CAD build for the part. Positions are in the model's coordinates, mm. A direction names the side the tool comes from. Give positions to 0.01 mm unless a question says otherwise; leave off trailing zeros. Order: outer loops, then holes, each group sorted by start corner. A loop starts at its lowest first (then second) coordinate and runs counter-clockwise, first axis right, second up. Notation, with made-up numbers: (71, 4) -> (79, 4) arc R18 cw to (79, 13) -> close; hole circle Ø2 at (43, -7.5). An arc over 180 degrees is marked (long way). Answer as CSV lines item,"result".
```python
from build123d import *

# Parameters (mm, degrees)
SKETCH_1_R          = 15
EXTRUDE_1_DEPTH     = 50
SKETCH_2_R          = 20
EXTRUDE_2_DEPTH     = 15
SKETCH_3_W          = 60.184655206
SKETCH_3_H          = 5
CUT_EXTRUDE_1_DEPTH = 5
CHAMFER_1_SIZE      = 1


with BuildPart() as part:
    # 草图1 → 凸台-拉伸1 (new, symmetric)
    with BuildSketch(Plane(origin=(0, 0, 0), x_dir=(1, 0, 0), z_dir=(0, 1, 0))):
        with Locations(Location((0, 0, 0), (0, 0, 270))):
            Circle(SKETCH_1_R)
    extrude(amount=EXTRUDE_1_DEPTH, both=True)

    # 草图2 → 凸台-拉伸2 (add)
    with BuildSketch(Plane(origin=(0, 50, 0), x_dir=(1, 0, 0), z_dir=(0, 1, 0))):
        with Locations(Location((0, 0, 0), (0, 0, 270))):
            Circle(SKETCH_2_R)
    extrude(amount=EXTRUDE_2_DEPTH)

    # 草图3 → 切除-拉伸1 (cut)
    with BuildSketch(Plane(origin=(0, 65, 0), x_dir=(1, 0, 0), z_dir=(0, 1, 0))):
        Rectangle(SKETCH_3_W, SKETCH_3_H)
    extrude(amount=-CUT_EXTRUDE_1_DEPTH, mode=Mode.SUBTRACT)

    # 倒角1
    chamfer_1_edges = [part.edges().sort_by_distance(p)[0] for p in [
        (0, -50, -15),
    ]]
    chamfer(chamfer_1_edges, length=CHAMFER_1_SIZE)


solid = part.part
```
1) Pin check, flat tips, straight feed: P1, Ø1.5, axis at x = -8.5, y = 62.5, coming from the -Z side; P2, Ø1.5, axis at y = 14.5, z = -12, coming from the +X side; P3, Ø5.5, axis at x = 3.5, z = -0.5, coming from the +Y side; P4, Ø8, axis at y = 13.5, z = 11, coming from the -X side. Stop position of each tip, or through.
Data:
P1,"stops at z = -18.44"
P2,"stops at x = 9.92"
P3,"stops at y = 65"
P4,"stops at x = -13.27"
2) Band-saw the part on A-A, the plane x = 0. Write the cut outline in (y, z), then the cut area to 3 significant figures.
Data:
outline,"(-50, -14) -> (-49, -15) -> (50, -15) -> (50, -20) -> (65, -20) -> (65, -2.5) -> (60, -2.5) -> (60, 2.5) -> (65, 2.5) -> (65, 20) -> (50, 20) -> (50, 15) -> (-49, 15) -> (-50, 14) -> close"
area,"3,570 mm2"
3) Which spindle directions (+Z, -Z, +X, -X, +Y, -Y) get a long thin tool onto all of the face, cutting with end or side? Do faces 1 (the flat face through (0, 65, -9)), 2 (the flat face through (15, 50, 3)), 3 (the flat face through (0, 63, -2.5)). Say none if no direction does.
Data:
face 1,"+Z, -Z, +X, -X, +Y"
face 2,"-Y"
face 3,"+X, -X, +Y"
4) Band-saw the part on B-B, the plane z = 0. Write the cut outline in (x, y), then the cut area to 3 significant figures.
Data:
outline,"(-20, 50) -> (-15, 50) -> (-15, -49) -> (-14, -50) -> (14, -50) -> (15, -49) -> (15, 50) -> (20, 50) -> (20, 60) -> (-20, 60) -> close"
area,"3,400 mm2"
5) Pull direction Z, two halves, no side cores. Call faces 4 (the cylindrical face through (0.66, 1.193, -14.985)), 5 (the flat face through (0, 63, 2.5)), 6 (the flat face through (0, 65, 9)): pulls with the +Z half, pulls with the -Z half, needs draft (parallel to the pull), parting line crosses it, or undercut.
Data:
face 4,"parting line crosses it"
face 5,"undercut"
face 6,"needs draft"
6) Wall check: line 1 along Y through (x, z) = (12, 1); line 2 along Y through (x, z) = (16.5, -5.5); line 3 along X through (y, z) = (-22.5, -3). Give the ranges that are in metal, low to high. Write a range as [from, to].
Data:
line 1,"y = [-50, 60]"
line 2,"y = [50, 65]"
line 3,"x = [-14.7, 14.7]"
7) Band-saw the part on C-C, the plane y = 14. Write the cut outline in (x, z), then the cut area to 3 significant figures.
Data:
outline,"circle Ø30 at (0, 0)"
area,"707 mm2"
8) Band-saw the part on D-D, the plane x = 17. Write the cut outline in (y, z).
Data:
outline,"(50, -10.54) -> (65, -10.54) -> (65, -2.5) -> (60, -2.5) -> (60, 2.5) -> (65, 2.5) -> (65, 10.54) -> (50, 10.54) -> close"
